Print and shaded views of the part. All mm, measured from the part's lowest x, y and z. A direction names the side the tool comes from. Round coordinates to 2 decimals unless told otherwise and drop trailing zeros. Write each loop counter-clockwise with the first axis right and the second up, starting at its lowest first coordinate (ties: lowest second). Pieces come first, ordered by that corner, then holes. Notation, with made-up numbers: M -16,-24 L 35,-24 A22 ccw 35,6 Z; hole C 10,5 d7. An arc over 180 degrees is marked long. Write item = value, one per line.
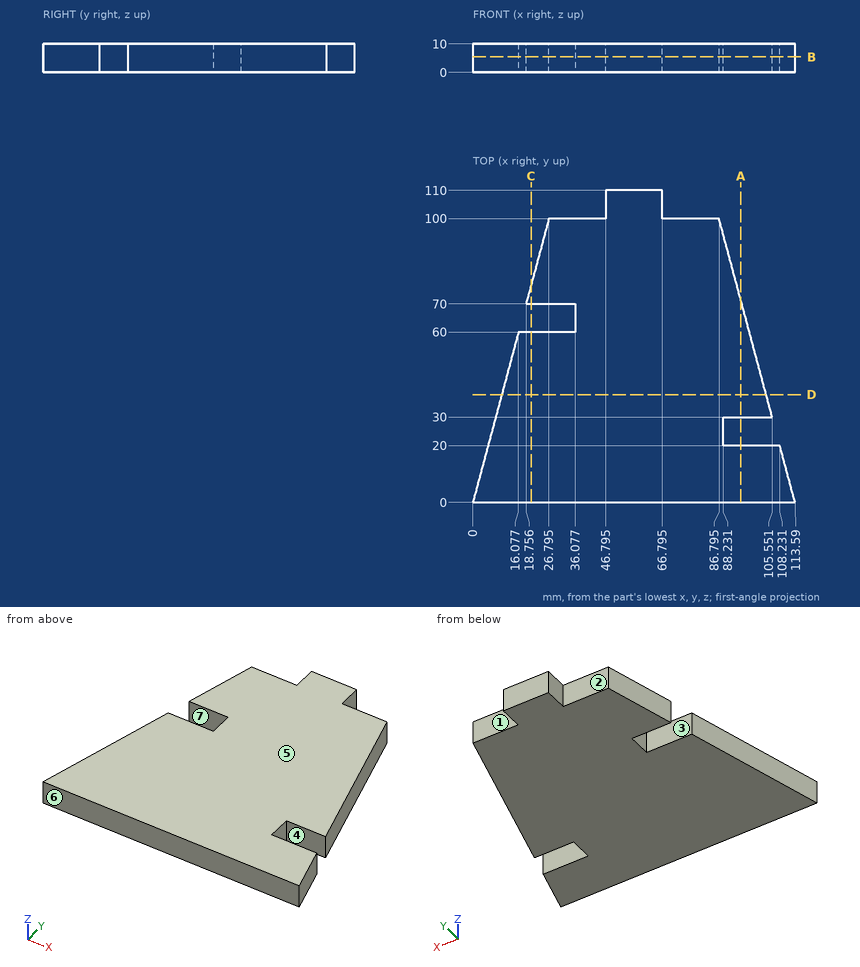
1. Tool access for the marked faces 1, 2, 3 and 4: list every direction of +Z, -Z, +X, -X, +Y, -Y with a clear straight run to the whole face (end or side of a thin tool).
Responses:
face_1 = +Z, -Z, +X, +Y
face_2 = +Z, -Z, -X, +Y
face_3 = +Z, -Z, -X
face_4 = +Z, -Z, +X
2. Band-saw the part on C-C (x = 20.5). List the corners of the cut face in (y, z).
Responses:
outline = M 0,0 L 60,0 L 60,10 L 0,10 Z; M 70,0 L 76.51,0 L 76.51,10 L 70,10 Z
3. Mould opens along Y. For the marked faces 5, 6 and 7 say: pulls with the +Y half, pulls with the -Y half, needs draft (parallel to the pull), parting line crosses it, or undercut.
Responses:
face_5 = needs draft
face_6 = pulls with the -Y half
face_7 = undercut
4. Probe probe 1 along Y at (x, z) = (31, 0.75); probe 2 along Y at (x, z) = (71, 4); probe 3 along X at (y, z) = (50, 3.75). List the from-to ranges inside material, lowest first.
Responses:
probe_1 = 0 to 60, 70 to 100
probe_2 = 0 to 100
probe_3 = 13.4 to 100.19
5. Band-saw the part on D-D (y = 38). List the corners of the cut face in (x, z), plus the area to 3 significant figures.
Responses:
outline = M 10.18,0 L 103.41,0 L 103.41,10 L 10.18,10 Z
area = 932 mm²
6. Band-saw the part on A-A (x = 94.5). List the corners of the cut face in (y, z) (1 decimal).
Responses:
outline = M 0,0 L 20,0 L 20,10 L 0,10 Z; M 30,0 L 71.2,0 L 71.2,10 L 30,10 Z
7. Flat gauge pins, fed straight in: pin 1 (3 mm diameter, centred on y = 23.5, z = 3.5, fed in from +X); pin 2 (6 mm diameter, centred on x = 15, z = 8, fed in from +Y); pin 3 (1.5 mm diameter, centred on y = 96, z = 8.5, fed in from -X). Where does each tip first touch, or does it go through?
Responses:
pin_1 = 88.23
pin_2 = 60
pin_3 = 25.52
8. Band-saw the part on B-B (z = 5.5). List the corners of the cut face in (x, y) (1 decimal), plus the area to 3 significant figures.
Responses:
outline = M 0,0 L 113.6,0 L 108.2,20 L 88.2,20 L 88.2,30 L 105.6,30 L 86.8,100 L 66.8,100 L 66.8,110 L 46.8,110 L 46.8,100 L 26.8,100 L 18.8,70 L 36.1,70 L 36.1,60 L 16.1,60 Z
area = 8,510 mm²
